```python
from build123d import *

# Parameters (mm, degrees)
SKETCH_1_R          = 3.5
EXTRUDE_1_DEPTH     = 30
FILLET_1_R          = 10
CUT_EXTRUDE_1_DEPTH = 30
SKETCH_3_W          = 18.572765592
SKETCH_3_H          = 9
SKETCH_3_W_2        = 28.522519482
CUT_EXTRUDE_2_DEPTH = 15


with BuildPart() as part:
    # 草图1 → 凸台-拉伸1 (new body)
    with BuildSketch(Plane.XY):
        with BuildLine():
            Line((-32.5, 1.5), (26.367564687, 1.5))
            ThreePointArc((26.367564687, 1.5), (34.720903057, 10.807641922), (32.5, -1.5))
            Line((32.5, -1.5), (-32.5, -1.5))
            Line((-32.5, -1.5), (-32.5, 1.5))
        make_face()
        with Locations((31.86456148, 4.96886527)):
            Circle(SKETCH_1_R, mode=Mode.SUBTRACT)
    extrude(amount=EXTRUDE_1_DEPTH)

    # 圆角1
    fillet_1_edges = [part.edges().sort_by_distance(p)[0] for p in [
        (-32.5, 0, 30),
        (-32.5, 0, 0),
    ]]
    fillet(fillet_1_edges, radius=FILLET_1_R)

    # 草图2 → 切除-拉伸1 (cut)
    with BuildSketch(Plane(origin=(0, 1.5, 0), x_dir=(1, 0, 0), z_dir=(0, 1, 0))):
        with BuildLine():
            Line((-22.5, -12.87764733), (7.5, -12.87764733))
            ThreePointArc((7.5, -12.87764733), (10, -15.37764733), (7.5, -17.87764733))
            Line((7.5, -17.87764733), (-22.5, -17.87764733))
            ThreePointArc((-22.5, -17.87764733), (-25, -15.37764733), (-22.5, -12.87764733))
        make_face()
    extrude(amount=-CUT_EXTRUDE_1_DEPTH, mode=Mode.SUBTRACT)

    # 草图3 → 切除-拉伸2 (cut, symmetric)
    with BuildSketch(Plane(origin=(0, 1.5, 0), x_dir=(1, 0, 0), z_dir=(0, 1, 0))):
        with Locations((34.650944276, -25.5)):
            Rectangle(SKETCH_3_W, SKETCH_3_H)
        with Locations((39.625821221, -4.5)):
            Rectangle(SKETCH_3_W_2, SKETCH_3_H)
    extrude(amount=CUT_EXTRUDE_2_DEPTH, both=True, mode=Mode.SUBTRACT)


solid = part.part
```
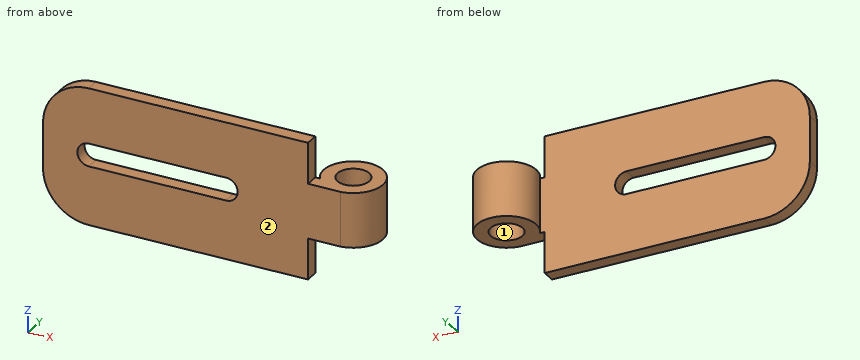
Verification items for the finished model (mm, model axes). Face numbers are marked on the shaded views. Coordinates: 2 decimals unless noted, no trailing zeros. Loops run counter-clockwise (first coordinate to the right, second up) from the corner with the lowest first, then second, coordinate; pieces in that order, holes last. Notation, with made-up numbers: (85.5, 0.5) -> (89.5, 0.5) arc R25 cw to (89.5, 14.5) -> close; hole circle Ø1 at (-9.5, -8.5). An arc over 180 degrees is marked (long way). Answer in a Markdown table with one row per item. Add a question column.
1. Draft check along X on the marked faces 1 and 2. Enter one of: +X half, -X half, draft (parallel to the pull), parting line (faces both ways), or undercut.
2. Section check C-C, the plane y = -0.5. Enter the section's corners in (x, z).
3. Section check A-A, the plane x = -18.5. Enter the section's corners in (y, z), then the cut area to 3 significant figures.
4. Depth check by flat-ended pin: P1, Ø12, axis at x = 28.5, z = 14, coming from the +Y side; P2, Ø0.9, axis at y = 0.5, z = 2.5, coming from the +X side; P3, Ø1, axis at y = 4, z = 18.5, coming from the +X side; P4, Ø4, axis at x = 32, y = 7, coming from the -Z side. Enter the tip coordinate at first touch or a pass-through.
5. Material ranges on probe 1 along Z at (x, y) = (29, 0.5); probe 2 along Y at (x, z) = (24, 13.75); probe 3 along X at (y, z) = (2.5, 15), recorded low to high. Write a range as [from, to].
6. Section check B-B, the plane y = 4.25. Enter the section's corners in (x, z), then the cut area to 3 significant figures.
7. Section check D-D, the plane x = 14.5. Enter the section's corners in (y, z), then the cut area to 3 significant figures.
Derived:
| question | item | result |
|---|---|---|
| 1 | face 1 | undercut |
| 1 | face 2 | draft |
| 2 | outline | (-32.5, 10) arc R10 ccw to (-22.5, 0) -> (25.36, 0) -> (25.36, 9) -> (35.38, 9) -> (35.38, 21) -> (25.36, 21) -> (25.36, 30) -> (-22.5, 30) arc R10 ccw to (-32.5, 20) -> close; hole (-22.5, 12.88) -> (7.5, 12.88) arc R2.5 ccw to (7.5, 17.88) -> (-22.5, 17.88) arc R2.5 ccw to start |
| 3 | outline | (-1.5, 0) -> (1.5, 0) -> (1.5, 12.88) -> (-1.5, 12.88) -> close; (-1.5, 17.88) -> (1.5, 17.88) -> (1.5, 30) -> (-1.5, 30) -> close |
| 3 | area | 75.0 mm² |
| 4 | P1 | stops at y = 11.47 |
| 4 | P2 | stops at x = 25.36 |
| 4 | P3 | stops at x = 38.35 |
| 4 | P4 | stops at z = 9 |
| 5 | probe 1 | z = [9, 21] |
| 5 | probe 2 | y = [-1.5, 1.5] |
| 5 | probe 3 | x = [25.85, 29.38], [34.35, 37.88] |
| 6 | outline | (25.4, 9) -> (28.44, 9) -> (28.44, 21) -> (25.4, 21) -> close; (35.29, 9) -> (38.32, 9) -> (38.32, 21) -> (35.29, 21) -> close |
| 6 | area | 72.8 mm² |
| 7 | outline | (-1.5, 0) -> (1.5, 0) -> (1.5, 30) -> (-1.5, 30) -> close |
| 7 | area | 90.0 mm² |
